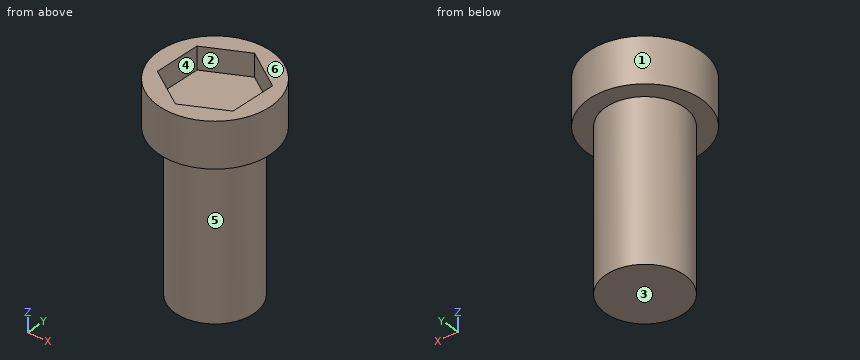
from build123d import *

# Parameters (mm, degrees)
SKETCH1_R           = 2.5
BOSS_EXTRUDE1_DEPTH = 2
CUT_EXTRUDE1_DEPTH  = 1
SKETCH3_R           = 1.75
BOSS_EXTRUDE2_DEPTH = 7


with BuildPart() as part:
    # Sketch1 → Boss-Extrude1 (new body)
    with BuildSketch(Plane.XY):
        Circle(SKETCH1_R)
    extrude(amount=BOSS_EXTRUDE1_DEPTH)

    # Sketch2 → Cut-Extrude1 (cut)
    with BuildSketch(Plane.XY.offset(2)):
        Polygon((1.663695781, -1.114955786), (1.797427926, 0.883324918), (0.133732144, 1.998280704), (-1.663695781, 1.114955786), (-1.797427926, -0.883324918), (-0.133732144, -1.998280704), align=None)
    extrude(amount=-CUT_EXTRUDE1_DEPTH, mode=Mode.SUBTRACT)

    # Sketch3 → Boss-Extrude2 (add)
    with BuildSketch(Plane(origin=(0, 0, 0), x_dir=(-1, 0, 0), z_dir=(0, 0, -1))):
        Circle(SKETCH3_R)
    extrude(amount=BOSS_EXTRUDE2_DEPTH)


solid = part.part
For this review, take the finished solid that the model builds, in its own axes (mm). Face numbers are marked on the shaded views. A direction names the side the tool comes from. Round coordinates to 2 decimals unless told otherwise and drop trailing zeros. Write each loop counter-clockwise with the first axis right and the second up, starting at its lowest first coordinate (ties: lowest second). Pieces come first, ordered by that corner, then holes. Notation, with made-up numbers: M 17,22 L 70,22 A15 ccw 70,51 Z; hole C -40,82 d3. An arc over 180 degrees is marked long. Write item = value, one per line. Start each with the question number.
(1) For line 1 along Z through (x, y) = (1.2, -1.95); line 2 along Z through (x, y) = (0.3, 1.55); line 3 along Y through (x, z) = (-0.2, 1.25), list the stretches that pass through material, from the lowest coordinate up.
(2) We need section A-A (y = 1.55). Give the boundary of the cut face in (x, z).
(3) For the marked faces 4, 5 and 6, list the 3-axis set-ups (+Z, -Z, +X, -X, +Y, -Y) from which the entire face can be reached by the end or side of a thin tool; tool diameter is ignored.
(4) The part is to be moulded in two halves that separate along Y. For the marked faces 1, 2 and 3, say which applies: +Y half, -Y half, draft (parallel to the pull), parting line (faces both ways), or undercut.
(5) Clearance check with flat-ended pins moving along their axes: pin 1 Ø2 at (y, z) = (-1.5, -6) entering from -X; pin 2 Ø1 at (x, z) = (-1, -3) entering from +Y; pin 3 Ø1 at (y, z) = (-1.5, -1) entering from +X. State where each tip first meets the part, or that it passes through.
(6) We need section B-B (x = -1.05). Give the boundary of the cut face in (y, z).
(7) We need section C-C (z = -1.75). Give the boundary of the cut face in (x, y), then the cut area to 3 significant figures.
Results found:
q1.line_1 = 0 to 2
q1.line_2 = -7 to 1
q1.line_3 = -2.49 to -1.95, 1.83 to 2.49
q2.outline = M -1.96,0 L -0.81,0 L -0.81,-7 L 0.81,-7 L 0.81,0 L 1.96,0 L 1.96,2 L 0.8,2 L 0.8,1 L -0.78,1 L -0.78,2 L -1.96,2 Z
q3.face_4 = +Z
q3.face_5 = -Z
q3.face_6 = +Z, +X, -X, +Y, -Y
q4.face_1 = parting line
q4.face_2 = undercut
q4.face_3 = draft
q5.pin_1 = -1.68
q5.pin_2 = 1.68
q5.pin_3 = 1.44
q6.outline = M -2.27,0 L -1.4,0 L -1.4,-7 L 1.4,-7 L 1.4,0 L 2.27,0 L 2.27,2 L 1.42,2 L 1.42,1 L -1.38,1 L -1.38,2 L -2.27,2 Z
q7.outline = C 0,0 d3.5
q7.area = 9.62 mm²
